Verification items for the finished model (mm, model axes). A direction names the side the tool comes from. Give positions to 0.01 mm unless a question says otherwise; leave off trailing zeros. Write each loop counter-clockwise with the first axis right and the second up, starting at its lowest first coordinate (ties: lowest second). Pieces come first, ordered by that corner, then holes. Notation, with made-up numbers: M 65.25,-29 L 82.25,-29 A13 cw 82.25,-17 Z; hole C -39.75,26 d10. An arc over 180 degrees is marked long. Answer as a JSON object with one key per item and string values.
```python
from build123d import *


with BuildPart() as part:
    # Sketch1 → Revolve1 (revolve)
    with BuildSketch(Plane.XY, mode=Mode.PRIVATE) as revolve1_sk:
        with BuildLine():
            Line((20, 22.5), (20, -22.5))
            Line((20, -22.5), (25, -22.5))
            Line((25, -22.5), (25, 4.5))
            Line((25, 4.5), (39.5, 4.5))
            ThreePointArc((39.5, 4.5), (44, 9), (39.5, 13.5))
            Line((39.5, 13.5), (25, 13.5))
            Line((25, 13.5), (25, 22.5))
            Line((25, 22.5), (20, 22.5))
        make_face()
    revolve(revolve1_sk.sketch.rotate(Axis((0, 22.5, 0), (0, -1, 0)), 180), axis=Axis((0, 22.5, 0), (0, -1, 0)))


solid = part.part
```
1) Section check B-B on z = 0. Record the boundary of the cut face in (x, y), and give its area (3 significant figures).
Completed:
{"outline": "M -39.5,4.5 L -25,4.5 L -25,-22.5 L -20,-22.5 L -20,22.5 L -25,22.5 L -25,13.5 L -39.5,13.5 A4.5 ccw Z; M 20,-22.5 L 25,-22.5 L 25,4.5 L 39.5,4.5 A4.5 ccw 39.5,13.5 L 25,13.5 L 25,22.5 L 20,22.5 Z", "area": "775 mm2"}
2) Section check C-C on y = 19. Record the boundary of the cut face in (x, z), and give its area (3 significant figures).
Completed:
{"outline": "C 0,0 d50; hole C 0,0 d40", "area": "707 mm2"}
3) Thickness scan on L1, parallel to Z at x = 0, y = -6.5; L2, parallel to Z at x = 13.5, y = 10.5; L3, parallel to X at y = -5, z = 12. Record the ranges inside material, lowest first.
Completed:
{"L1": "z = -25 to -20, 20 to 25", "L2": "z = -41.61 to -14.76, 14.76 to 41.61", "L3": "x = -21.93 to -16, 16 to 21.93"}
4) Release check for a two-part mould opening along X. For faces 1 (the face through (19.98, -0.32, -0.88)), 2 (the face through (-23.846, -8.811, -7.509)), 3 (the face through (-1, 4.5, 26)) record: pulls with the +X half, pulls with the -X half, needs draft (parallel to the pull), parting line crosses it, or undercut.
Completed:
{"face 1": "undercut", "face 2": "parting line crosses it", "face 3": "needs draft"}
5) Section check A-A on x = 0. Record the boundary of the cut face in (y, z), and give its area (3 significant figures).
Completed:
{"outline": "M -22.5,-25 L 4.5,-25 L 4.5,-39.5 A4.5 ccw 13.5,-39.5 L 13.5,-25 L 22.5,-25 L 22.5,-20 L -22.5,-20 Z; M -22.5,20 L 22.5,20 L 22.5,25 L 13.5,25 L 13.5,39.5 A4.5 ccw 4.5,39.5 L 4.5,25 L -22.5,25 Z", "area": "775 mm2"}
6) Go/stop test with flat-tipped pins: pin 1 (10 mm diameter, centred on y = 9, z = -9.5, fed in from -X); pin 2 (4 mm diameter, centred on x = 13.5, y = -17, fed in from -Z); pin 3 (12 mm diameter, centred on x = 31.5, y = -6, fed in from +Z); pin 4 (3 mm diameter, centred on y = 11.5, z = -18.5, fed in from -X). Record where each tip stops, or that it passes through.
Completed:
{"pin 1": "stops at x = -43.77", "pin 2": "stops at z = -22.2", "pin 3": "passes through", "pin 4": "stops at x = -40.14"}
7) Section check D-D on y = 11. Record the boundary of the cut face in (x, z).
Completed:
{"outline": "C 0,0 d87.06; hole C 0,0 d40"}
8) Access from +Z, -Z, +X, -X, +Y, -Y to the whole of each face (thin tool, end or side, straight path). Record for faces 4 (the face through (-23.846, 18.063, -7.509)), 5 (the face through (11, 22.5, -17)).
Completed:
{"face 4": "+Y", "face 5": "+Z, -Z, +X, -X, +Y"}
